For this review, take the finished solid that the model builds, in its own axes (mm). Round coordinates to 2 decimals unless told otherwise and drop trailing zeros. Loops run counter-clockwise (first coordinate to the right, second up) from the corner with the lowest first, then second, coordinate; pieces in that order, holes last.
1. Consider section A-A on y = 5.25. State the section outline as (x, z) points.
2. Clearance check with flat-ended pins moving along their axes: pin 1 Ø9 at (x, z) = (10.5, 334.5) entering from +Y; pin 2 Ø10 at (x, z) = (11.5, 215) entering from +Y. State where each tip first meets the part, or that it passes through.
3. To check wall thickness, follow line 1 along X through (y, z) = (18.75, 35); line 2 along X through (y, z) = (4, 335); line 3 along Y through (x, z) = (14.5, 92.5). State the ranges of each line that lie inside material, in increasing order.
from build123d import *

# Parameters (mm, degrees)
SKETCH_1_W                   = 23
SKETCH_1_H                   = 22
EXTRUDE_1_DEPTH              = 430
HOLE_WIZARD_M6_1_D           = 6.6
HOLE_WIZARD_M6_1_CBORE_D     = 11
HOLE_WIZARD_M6_1_CBORE_DEPTH = 6.4
PATTERN_LINEAR_1_COUNT       = 7
PATTERN_LINEAR_1_PITCH       = 60


with BuildPart() as part:
    # 草图1 → 凸台-拉伸1 (new body)
    with BuildSketch(Plane.XY):
        with Locations((11.5, 11)):
            Rectangle(SKETCH_1_W, SKETCH_1_H)
    extrude(amount=EXTRUDE_1_DEPTH)

    # M6 六角凹头螺钉的柱形沉头孔1 (through all)
    with Locations(Plane(origin=(0, 22, 0), x_dir=(1, 0, 0), z_dir=(0, 1, 0))):
        with Locations((11.5, -395)):
            hole_wizard_m6_1 = CounterBoreHole(HOLE_WIZARD_M6_1_D / 2, HOLE_WIZARD_M6_1_CBORE_D / 2, HOLE_WIZARD_M6_1_CBORE_DEPTH)

    # 阵列(线性)1: M6 六角凹头螺钉的柱形沉头孔1 ×7
    with Locations(*[(0, 0, -i * PATTERN_LINEAR_1_PITCH) for i in range(1, PATTERN_LINEAR_1_COUNT)]):
        add(hole_wizard_m6_1, mode=Mode.SUBTRACT)


solid = part.part
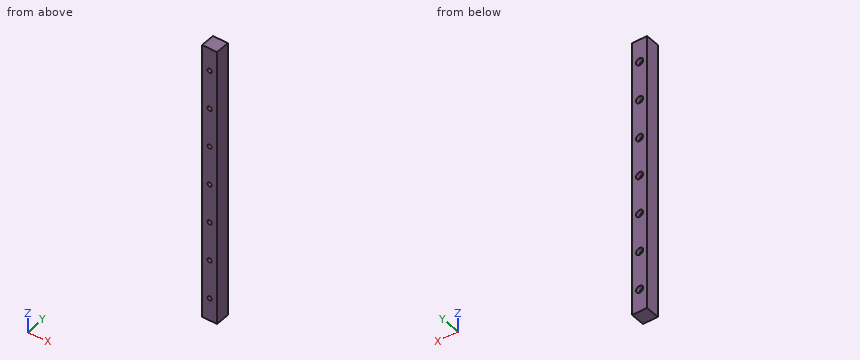
Resolved:
1. outline: (0, 0) - (23, 0) - (23, 430) - (0, 430) - close; hole circle Ø6.6 at (11.5, 35); hole circle Ø6.6 at (11.5, 95); hole circle Ø6.6 at (11.5, 155); hole circle Ø6.6 at (11.5, 215); hole circle Ø6.6 at (11.5, 275); hole circle Ø6.6 at (11.5, 335); hole circle Ø6.6 at (11.5, 395)
2. pin 1: stops at y = 22
2. pin 2: stops at y = 15.6
3. line 1: x = 0 to 6, 17 to 23
3. line 2: x = 0 to 8.2, 14.8 to 23
3. line 3: y = 0 to 15.6
